Work out the finished part from the listing and answer in its coordinate system (mm). A direction names the side the tool comes from. Round coordinates to 2 decimals unless told otherwise and drop trailing zeros. Order: outer loops, then holes, each group sorted by start corner. A loop starts at its lowest first (then second) coordinate and runs counter-clockwise, first axis right, second up. Notation, with made-up numbers: (-1, 46.5) -> (4, 46.5) arc R14 ccw to (4, 67.5) -> close; hole circle Ø6 at (-25.5, 12.5). An arc over 180 degrees is marked (long way). Use a Markdown table: item, result. Add a question column.
Item 1: A cutting plane is placed at C-C, the plane y = 8. Give the number of separate pieces and of enclosed holes in the cut face, plus the area to 3 significant figures.
Item 2: A cutting plane is placed at B-B, the plane x = -78.5. Determine the outline of the cut face in (y, z), plus the area to 3 significant figures.
Item 3: Find the intervals of material crossed by L1, parallel to Z at x = -12.5, y = 2.35; L2, parallel to X at y = 3.25, z = 77.5; L3, parallel to Z at x = 31, y = 2.5, in increasing order. Write a range as [from, to].
Item 4: Flat-ended cylindrical pins translate along their axes: P1, Ø2.5, axis at x = -12.5, z = -22.5, coming from the -Y side; P2, Ø9, axis at x = -78, z = 58, coming from the +Y side; P3, Ø5, axis at x = 12.5, z = -22.5, coming from the +Y side. Find the tip coordinate at first contact, or state that the pin passes through.
Item 5: A tool of negligible diameter and unlimited length cuts with its end or side. For faces 4 (the cylindrical face through (-84, 7, 58)), 5 (the flat face through (123, 5, 97)), from which of +Z, -Z, +X, -X, +Y, -Y can it reach the whole face along a straight path? Write none if from no direction.
Item 6: A cutting plane is placed at A-A, the plane x = -45. Determine the outline of the cut face in (y, z).
Item 7: For a pull along X with two mould halves and no side action, classify faces 1 (the flat face through (-2, 5, -100)), 2 (the flat face through (-1, 5, -90)), 3 (the flat face through (-125, 5, 1)) as +X half, -X half, draft (parallel to the pull), parting line (faces both ways), or undercut.
from build123d import *

# Parameters (mm, degrees)
SKETCH1_W                                            = 250
SKETCH1_H                                            = 200
BOSS_EXTRUDE1_DEPTH                                  = 10
M6_TAPPED_HOLE1_D                                    = 5
M6_TAPPED_HOLE1_DEPTH                                = 17
M6_TAPPED_HOLE1_TIP                                  = 1.502151548
SKETCH6_W                                            = 110
SKETCH6_H                                            = 50
CUT_EXTRUDE2_DEPTH                                   = 161.390149323
FILLET1_R                                            = 3
CHAMFER1_SIZE                                        = 5
CBORE_FOR_M6_HEXAGON_SOCKET_HEAD_CAP_SCR_D           = 6.6
CBORE_FOR_M6_HEXAGON_SOCKET_HEAD_CAP_SCR_CBORE_D     = 11
CBORE_FOR_M6_HEXAGON_SOCKET_HEAD_CAP_SCR_CBORE_DEPTH = 6.8
CBORE_FOR_M4_HEXAGON_SOCKET_HEAD_CAP_SCR_D           = 4.5
CBORE_FOR_M4_HEXAGON_SOCKET_HEAD_CAP_SCR_CBORE_D     = 8
CBORE_FOR_M4_HEXAGON_SOCKET_HEAD_CAP_SCR_CBORE_DEPTH = 4.6


with BuildPart() as part:
    # Sketch1 → Boss-Extrude1 (new body)
    with BuildSketch(Plane(origin=(0, 0, 0), x_dir=(1, 0, 0), z_dir=(0, 1, 0))):
        Rectangle(SKETCH1_W, SKETCH1_H)
    extrude(amount=BOSS_EXTRUDE1_DEPTH)

    # M6 Tapped Hole1
    with Locations(Plane(origin=(0, 10, 0), x_dir=(1, 0, 0), z_dir=(0, 1, 0))):
        with Locations((105, -77.5), (-100, -77.5), (-100, 17.5), (105, 17.5), (-100, 37.5), (-100, 67.5), (105, 37.5), (105, 67.5), (-100, -57.5), (-100, -27.5), (105, -57.5), (105, -27.5)):
            Hole(M6_TAPPED_HOLE1_D / 2, depth=M6_TAPPED_HOLE1_DEPTH)
            with Locations((0, 0, -(M6_TAPPED_HOLE1_DEPTH + M6_TAPPED_HOLE1_TIP / 2))):  # 118° drill point
                Cone(0, M6_TAPPED_HOLE1_D / 2, M6_TAPPED_HOLE1_TIP, mode=Mode.SUBTRACT)

    # Sketch6 → Cut-Extrude2 (cut, through all)
    with BuildSketch(Plane(origin=(0, 10, 0), x_dir=(1, 0, 0), z_dir=(0, 1, 0))):
        with Locations((0, 65)):
            Rectangle(SKETCH6_W, SKETCH6_H)
    extrude(amount=-CUT_EXTRUDE2_DEPTH, mode=Mode.SUBTRACT)

    # Fillet1
    fillet1_edges = [part.edges().sort_by_distance(p)[0] for p in [
        (-55, 5, -40),
        (-55, 5, -90),
        (55, 5, -90),
        (55, 5, -40),
    ]]
    fillet(fillet1_edges, radius=FILLET1_R)

    # Chamfer1
    chamfer1_edges = [part.edges().sort_by_distance(p)[0] for p in [
        (125, 5, 100),
        (-125, 5, 100),
        (-125, 5, -100),
        (125, 5, -100),
    ]]
    chamfer(chamfer1_edges, length=CHAMFER1_SIZE)

    # CBORE for M6 Hexagon socket head cap screws1 (through all)
    with Locations(Plane(origin=(0, 10, 0), x_dir=(1, 0, 0), z_dir=(0, 1, 0))):
        with Locations((-78.5, 58), (78.5, 58), (78.5, -58), (-78.5, -58)):
            CounterBoreHole(CBORE_FOR_M6_HEXAGON_SOCKET_HEAD_CAP_SCR_D / 2, CBORE_FOR_M6_HEXAGON_SOCKET_HEAD_CAP_SCR_CBORE_D / 2, CBORE_FOR_M6_HEXAGON_SOCKET_HEAD_CAP_SCR_CBORE_DEPTH)

    # CBORE for M4 Hexagon socket head cap screws1 (through all)
    with Locations(Plane(origin=(0, 10, 0), x_dir=(1, 0, 0), z_dir=(0, 1, 0))):
        with Locations((-12.5, 22.5), (12.5, 22.5), (12.5, -22.5), (-12.5, -22.5)):
            CounterBoreHole(CBORE_FOR_M4_HEXAGON_SOCKET_HEAD_CAP_SCR_D / 2, CBORE_FOR_M4_HEXAGON_SOCKET_HEAD_CAP_SCR_CBORE_D / 2, CBORE_FOR_M4_HEXAGON_SOCKET_HEAD_CAP_SCR_CBORE_DEPTH)


solid = part.part
Reported:
| question | item | result |
|---|---|---|
| 1 | separate pieces | 1 |
| 1 | enclosed holes | 21 |
| 1 | area | 43,600 mm² |
| 2 | outline | (0, -100) -> (10, -100) -> (10, -63.5) -> (3.2, -63.5) -> (3.2, -61.3) -> (0, -61.3) -> close; (0, -54.7) -> (3.2, -54.7) -> (3.2, -52.5) -> (10, -52.5) -> (10, 52.5) -> (3.2, 52.5) -> (3.2, 54.7) -> (0, 54.7) -> close; (0, 61.3) -> (3.2, 61.3) -> (3.2, 63.5) -> (10, 63.5) -> (10, 100) -> (0, 100) -> close |
| 2 | area | 1,810 mm² |
| 3 | L1 | [-100, -90], [-40, -24.75], [-20.25, 20.25], [24.75, 100] |
| 3 | L2 | [-125, -102.5], [-97.5, 102.5], [107.5, 125] |
| 3 | L3 | [-100, -90], [-40, 100] |
| 4 | P1 | through |
| 4 | P2 | y = 3.2 |
| 4 | P3 | y = 5.4 |
| 5 | face 4 | +Y |
| 5 | face 5 | +Z, +X, +Y, -Y |
| 6 | outline | (0, -100) -> (10, -100) -> (10, -90) -> (0, -90) -> close; (0, -40) -> (10, -40) -> (10, 100) -> (0, 100) -> close |
| 7 | face 1 | draft |
| 7 | face 2 | undercut |
| 7 | face 3 | -X half |
